For this review, take the finished solid that the model builds, in its own axes (mm). Coordinates: 2 decimals unless noted, no trailing zeros. Loops run counter-clockwise (first coordinate to the right, second up) from the corner with the lowest first, then second, coordinate; pieces in that order, holes last. Notation, with made-up numbers: (4, 75.5) - (12, 75.5) arc R16 ccw to (12, 83.5) - close; hole circle Ø10 at (89, -31). An arc over 180 degrees is marked (long way). One line per item, written item: value. Start each with the question number.
1. Take a section at C-C, the plane y = 8.25. State the section outline as (x, z) points.
2. Take a section at D-D, the plane y = 26. State the section outline as (x, z) points, and give its area (3 significant figures).
3. To check wall thickness, follow line 1 (X direction, y = 16.5, z = 1); line 2 (X direction, y = 10.25, z = 0); line 3 (Z direction, x = -25.5, y = 5.75). State the ranges of each line that lie inside material, in increasing order. Write a range as from..to.
4. Take a section at A-A, the plane x = 0. State the section outline as (y, z) points.
5. Take a section at B-B, the plane z = 0. State the section outline as (x, y) points, and give its area (3 significant figures).
6. The part is to be moulded in two halves that separate along Z. For faces 1 (the face through (33.71, 22.6, -4.43)), 2 (the face through (-2, 0, 32)), 3 (the face through (-2, 15, -75)), 4 (the face through (-23, 15, 23)), say which applies: released by +Z, released by -Z, zero draft, split by the parting line, or undercut.
```python
from build123d import *

# Parameters (mm, degrees)
SKETCH_1_W          = 310
SKETCH_1_H          = 150
EXTRUDE_1_DEPTH     = 30
SKETCH_2_R          = 31.75
CUT_EXTRUDE_1_DEPTH = 175.785582929
SKETCH_3_R          = 34
CUT_EXTRUDE_2_DEPTH = 15


with BuildPart() as part:
    # 草图1 → 凸台-拉伸1 (new body)
    with BuildSketch(Plane(origin=(0, 0, 0), x_dir=(1, 0, 0), z_dir=(0, 1, 0))):
        Rectangle(SKETCH_1_W, SKETCH_1_H)
    extrude(amount=EXTRUDE_1_DEPTH)

    # 草图2 → 切除-拉伸1 (cut, through all)
    with BuildSketch(Plane(origin=(0, 30, 0), x_dir=(1, 0, 0), z_dir=(0, 1, 0))):
        with Locations(Location((0, 0, 0), (0, 0, 270))):
            Circle(SKETCH_2_R)
    extrude(amount=-CUT_EXTRUDE_1_DEPTH, mode=Mode.SUBTRACT)

    # 草图3 → 切除-拉伸2 (cut)
    with BuildSketch(Plane(origin=(0, 30, 0), x_dir=(1, 0, 0), z_dir=(0, 1, 0))):
        with Locations(Location((0, 0, 0), (0, 0, 270))):
            Circle(SKETCH_3_R)
    extrude(amount=-CUT_EXTRUDE_2_DEPTH, mode=Mode.SUBTRACT)


solid = part.part
```
Solutions:
1. outline: (-155, -75) - (155, -75) - (155, 75) - (-155, 75) - close; hole circle Ø63.5 at (0, 0)
2. outline: (-155, -75) - (155, -75) - (155, 75) - (-155, 75) - close; hole circle Ø68 at (0, 0)
2. area: 42,900 mm2
3. line 1: -155..-33.99, 33.99..155
3. line 2: -155..-31.75, 31.75..155
3. line 3: -75..-18.92, 18.92..75
4. outline: (0, -75) - (30, -75) - (30, -34) - (15, -34) - (15, -31.75) - (0, -31.75) - close; (0, 31.75) - (15, 31.75) - (15, 34) - (30, 34) - (30, 75) - (0, 75) - close
5. outline: (-155, 0) - (-31.75, 0) - (-31.75, 15) - (-34, 15) - (-34, 30) - (-155, 30) - close; (31.75, 0) - (155, 0) - (155, 30) - (34, 30) - (34, 15) - (31.75, 15) - close
5. area: 7,330 mm2
6. face 1: undercut
6. face 2: zero draft
6. face 3: released by -Z
6. face 4: undercut
